from build123d import *

# Parameters (mm, degrees)
SKETCH1_R           = 60
BOSS_EXTRUDE1_DEPTH = 20
FILLET1_R           = 3
SKETCH2_R           = 10
BOSS_EXTRUDE2_DEPTH = 25
BOSS_EXTRUDE3_START = 25
SKETCH3_R           = 10
BOSS_EXTRUDE3_DEPTH = 25


with BuildPart() as part:
    # Sketch1 → Boss-Extrude1 (new body)
    with BuildSketch(Plane.XY):
        Circle(SKETCH1_R)
    extrude(amount=BOSS_EXTRUDE1_DEPTH)

    # Fillet1
    fillet1_edges = [part.edges().sort_by_distance(p)[0] for p in [
        (-60, 0, 0),
        (-60, 0, 20),
    ]]
    fillet(fillet1_edges, radius=FILLET1_R)

    # Sketch2 → Boss-Extrude2 (add)
    with BuildSketch(Plane(origin=(0, 0, 0), x_dir=(-1, 0, 0), z_dir=(0, 0, -1))):
        with Locations(Location((0, 0, 0), (0, 0, 180))):
            Circle(SKETCH2_R)
    extrude(amount=BOSS_EXTRUDE2_DEPTH)

    # Sketch3 → Boss-Extrude3 (add)
    with BuildSketch(Plane.XY.offset(20).offset(BOSS_EXTRUDE3_START)):
        Circle(SKETCH3_R)
    extrude(amount=-BOSS_EXTRUDE3_DEPTH)


solid = part.part
CAD build for the part. Positions are in the model's coordinates, mm. A direction names the side the tool comes from. Give positions to 0.01 mm unless a question says otherwise; leave off trailing zeros. Write each loop counter-clockwise with the first axis right and the second up, starting at its lowest first coordinate (ties: lowest second). Pieces come first, ordered by that corner, then holes. Notation, with made-up numbers: (86, 80) - (134, 80) arc R5 ccw to (134, 89) - close; hole circle Ø6 at (33, 18). An arc over 180 degrees is marked (long way). Answer as CSV lines item,"result".
Q1. Flat gauge pins, fed straight in: pin 1 Ø3 at (x, z) = (-19, 22.5) entering from +Y; pin 2 Ø6 at (x, z) = (-4, 13.5) entering from -Y; pin 3 Ø2 at (y, z) = (-23, 19.5) entering from +X; pin 4 Ø8 at (x, z) = (-11, 35) entering from +Y. Where does each tip first touch, or does it go through?
Result set:
pin 1,"through"
pin 2,"y = -59.99"
pin 3,"x = 55.1"
pin 4,"y = 7.14"
Q2. Band-saw the part on C-C (z = 40). Give the cut face in (x, y), and give its area (3 significant figures).
Result set:
outline,"circle Ø20 at (0, 0)"
area,"314 mm²"
Q3. 3-axis set-ups, long thin cutter, end or side, ignore diameter. For faces 1 (the face through (0, 0, -25)), 2 (the face through (-2.17, -9.76, 32.67)), 3 (the face through (-10, 0, -12)): which of +Z, -Z, +X, -X, +Y, -Y reach the whole face in a straight line?
Result set:
face 1,"-Z, +X, -X, +Y, -Y"
face 2,"+Z"
face 3,"-Z"
Q4. Drill centre lines: line 1 (Z direction, x = 3, y = 20); line 2 (Y direction, x = 31, z = 9.5); line 3 (X direction, y = 23.5, z = 0.5). Where is each one in solid material? Low to high. Write a range as from..to.
Result set:
line 1,"0..20"
line 2,"-51.37..51.37"
line 3,"-53.75..53.75"
Q5. Band-saw the part on A-A (y = 0). Give the cut face in (x, z), and give its area (3 significant figures).
Result set:
outline,"(-60, 3) arc R3 ccw to (-57, 0) - (-10, 0) - (-10, -25) - (10, -25) - (10, 0) - (57, 0) arc R3 ccw to (60, 3) - (60, 17) arc R3 ccw to (57, 20) - (10, 20) - (10, 45) - (-10, 45) - (-10, 20) - (-57, 20) arc R3 ccw to (-60, 17) - close"
area,"3,390 mm²"
